The model under review builds one solid part; all positions refer to its coordinate system, in mm. A direction names the side the tool comes from. Round coordinates to 2 decimals unless told otherwise and drop trailing zeros. Write each loop counter-clockwise with the first axis right and the second up, starting at its lowest first coordinate (ties: lowest second). Pieces come first, ordered by that corner, then holes. Notation, with made-up numbers: (4, 67.25) -> (20, 67.25) arc R12 ccw to (20, 87.25) -> close; hole circle Ø5 at (80.5, -8.5). An arc over 180 degrees is marked (long way). Answer in a Markdown table with one row per item. Add a question column.
```python
from build123d import *

# Parameters (mm, degrees)
SKETCH_1_R          = 24
SKETCH_1_R_2        = 20
EXTRUDE_1_DEPTH     = 15
SKETCH_2_W          = 20.6
SKETCH_2_H          = 3
SKETCH_2_W_2        = 4.5
SKETCH_5_W          = 3.1
SKETCH_5_H          = 3
CUT_EXTRUDE_1_DEPTH = 7
SKETCH_6_R          = 4
CUT_EXTRUDE_2_DEPTH = 38.107950631
CHAMFER_1_SIZE      = 1


with BuildPart() as part:
    # 草图1 → 凸台-拉伸1 (new, symmetric)
    with BuildSketch(Plane(origin=(0, 0, 0), x_dir=(1, 0, 0), z_dir=(0, 1, 0))):
        with Locations(Location((0, 0, 0), (0, 0, 270))):
            Circle(SKETCH_1_R)
        with Locations(Location((0, 0, 0), (0, 0, 270))):
            Circle(SKETCH_1_R_2, mode=Mode.SUBTRACT)
    extrude(amount=EXTRUDE_1_DEPTH, both=True)

    # 草图2 → 切除-旋转1 (revolve, cut)
    with BuildSketch(Plane.XY, mode=Mode.PRIVATE) as cut_revolve_1_sk:
        with Locations((10.3, 8.5)):
            Rectangle(SKETCH_2_W, SKETCH_2_H)
        with Locations((10.3, -8.5)):
            Rectangle(SKETCH_2_W, SKETCH_2_H)
        with Locations((25.25, 0)):
            Rectangle(SKETCH_2_W_2, SKETCH_2_H)
    revolve(cut_revolve_1_sk.sketch.rotate(Axis((0, 33.887302741, 0), (0, -1, 0)), 180), axis=Axis((0, 33.887302741, 0), (0, -1, 0)), mode=Mode.SUBTRACT)

    # 草图5 → 切除-拉伸1 (cut, symmetric)
    with BuildSketch(Plane(origin=(0, 0, 0), x_dir=(1, 0, 0), z_dir=(0, 1, 0))):
        with Locations((19.05, 0)):
            Rectangle(SKETCH_5_W, SKETCH_5_H)
        with Locations((-19.05, 0)):
            Rectangle(SKETCH_5_W, SKETCH_5_H)
    extrude(amount=CUT_EXTRUDE_1_DEPTH, both=True, mode=Mode.SUBTRACT)

    # 草图6 → 切除-拉伸2 (cut, through all)
    with BuildSketch(Plane(origin=(0, 0, 0), x_dir=(0, 0, -1), z_dir=(1, 0, 0))):
        with Locations(Location((0, 0, 0), (0, 0, 22.024312837))):
            Circle(SKETCH_6_R)
    extrude(amount=-CUT_EXTRUDE_2_DEPTH, mode=Mode.SUBTRACT)

    # 倒角1
    chamfer_1_edges = [part.edges().sort_by_distance(p)[0] for p in [
        (0, -15, -20),
        (0, 15, -20),
    ]]
    chamfer(chamfer_1_edges, length=CHAMFER_1_SIZE)


solid = part.part
```
1. For L1, parallel to Y at x = 22.5, z = 8; L2, parallel to Z at x = 0, y = -12.85, list the stretches that pass through material, from the lowest coordinate up.
2. Mouldability with a two-part tool opening along Y and no side actions: class faces 1 (the cylindrical face through (-19.524, -12.028, -4.336)), 2 (the cylindrical face through (16.35, 8.52, 12.53)) as pulls with the +Y half, pulls with the -Y half, needs draft (parallel to the pull), parting line crosses it, or undercut.
3. Tool access review of faces 3 (the cylindrical face through (0, 0, -20)), 4 (the flat face through (-17, -10, -11)): name each direction out of +Z, -Z, +X, -X, +Y, -Y from which nothing blocks a thin tool from reaching the whole face with its end or side.
4. Add section A-A on y = -5.5. Write out the cut boundary in (x, z).
5. Insertion check: pin 1 Ø1 at (x, y) = (-18, 4.5) entering from +Z; pin 2 Ø12 at (x, z) = (8, 8.5) entering from -Y; pin 3 Ø6 at (x, y) = (17.5, -5) entering from +Z; pin 4 Ø1.5 at (y, z) = (1, 0) entering from -X. Each pin has a flat end and moves straight along its axis. Give the tip position at first contact, or say it passes through.
6. Add section B-B on y = 0. Write out the cut boundary in (x, z), plus the area to 3 significant figures.
Filled in:
| question | item | result |
|---|---|---|
| 1 | L1 | -15 to -1.5, 1.5 to 15 |
| 1 | L2 | -24 to -20, 20 to 24 |
| 2 | face 1 | needs draft |
| 2 | face 2 | undercut |
| 3 | face 3 | +Y, -Y |
| 3 | face 4 | none |
| 4 | outline | circle Ø48 at (0, 0); hole (-20.6, -1.5) -> (-19.94, -1.5) arc R20 ccw to (19.94, -1.5) -> (20.6, -1.5) -> (20.6, 1.5) -> (19.94, 1.5) arc R20 ccw to (-19.94, 1.5) -> (-20.6, 1.5) -> close |
| 5 | pin 1 | z = 16.42 |
| 5 | pin 2 | through |
| 5 | pin 3 | z = 19.12 |
| 5 | pin 4 | x = 20.6 |
| 6 | outline | (-22.65, -4) arc R23 ccw (long way) to (-22.65, 4) -> (-19.6, 4) arc R20 cw to (19.94, 1.5) -> (20.6, 1.5) -> (20.6, -1.5) -> (19.94, -1.5) arc R20 cw to (-19.6, -4) -> close |
| 6 | area | 379 mm² |
